CAD build for the part. Positions are in the model's coordinates, mm. Give positions to 0.01 mm unless a question says otherwise; leave off trailing zeros. Write each loop counter-clockwise with the first axis right and the second up, starting at its lowest first coordinate (ties: lowest second). Pieces come first, ordered by that corner, then holes. Notation, with made-up numbers: (1, 15) - (22, 15) arc R31 cw to (22, 43) - close; hole circle Ø1 at (25, 86). An arc over 180 degrees is marked (long way). Answer as a JSON object with one key per item and string values.
from build123d import *

# Parameters (mm, degrees)
SKETCH1_W                  = 240
SKETCH1_H                  = 480
BOSS_EXTRUDE1_DEPTH        = 16
F_18_0_18_DIAMETER_HOLE1_D = 18


with BuildPart() as part:
    # Sketch1 → Boss-Extrude1 (new body)
    with BuildSketch(Plane(origin=(0, 0, 0), x_dir=(1, 0, 0), z_dir=(0, 1, 0))):
        Rectangle(SKETCH1_W, SKETCH1_H)
    extrude(amount=BOSS_EXTRUDE1_DEPTH)

    # Ø18.0 (18) Diameter Hole1 (through all)
    with Locations(Plane(origin=(0, 16, 0), x_dir=(1, 0, 0), z_dir=(0, 1, 0))):
        with Locations((-80, -215), (80, -215), (80, 215), (-80, 215)):
            Hole(F_18_0_18_DIAMETER_HOLE1_D / 2)


solid = part.part
Item 1: Cut at B-B (z = 215). Give the cut face in (x, y), and give its area (3 significant figures).
Entries:
{"outline": "(-120, 0) - (-89, 0) - (-89, 16) - (-120, 16) - close; (-71, 0) - (71, 0) - (71, 16) - (-71, 16) - close; (89, 0) - (120, 0) - (120, 16) - (89, 16) - close", "area": "3,260 mm2"}
Item 2: Cut at A-A (x = -80). Give the cut face in (y, z).
Entries:
{"outline": "(0, -240) - (16, -240) - (16, -224) - (0, -224) - close; (0, -206) - (16, -206) - (16, 206) - (0, 206) - close; (0, 224) - (16, 224) - (16, 240) - (0, 240) - close"}
Item 3: Probe line 1 (X direction, y = 5.5, z = 215); line 2 (Z direction, x = 80, y = 4.25); line 3 (X direction, y = 11.25, z = 216.5). List the from-to ranges inside material, lowest first. Write a range as from..to.
Entries:
{"line 1": "-120..-89, -71..71, 89..120", "line 2": "-240..-224, -206..206, 224..240", "line 3": "-120..-88.87, -71.13..71.13, 88.87..120"}
Item 4: Mould opens along X. For faces 1 (the cylindrical face through (75.16, 7.89, 207.41)), 2 (the flat face through (-2, 8, -240)), 3 (the flat face through (-120, 8, 3)) say: +X half, -X half, draft (parallel to the pull), parting line (faces both ways), or undercut.
Entries:
{"face 1": "undercut", "face 2": "draft", "face 3": "-X half"}
